```python
from build123d import *

# Parameters (mm, degrees)
SQUARE_FLANGE_SKETCH_70X70_W            = 70
SQUARE_FLANGE_SKETCH_70X70_H            = 70
SQUARE_MOUNTING_FLANGE_DEPTH            = 10
SQUARE_FLANGE_CORNER_FILLETS_R10_R      = 10
SQUARE_FLANGE_HOLES_SKETCH_R            = 5
SQUARE_FLANGE_MOUNTING_HOLES_4X_DEPTH   = 10
ROUND_FLANGE_HOLE_SKETCH_R              = 6
ROUND_FLANGE_BOLT_HOLE_12_DEPTH         = 229.350607619
ROUND_FLANGE_BOLT_HOLE_PATTERN_4X_COUNT = 4


with BuildPart() as part:
    # Housing Profile Sketch → Housing Body Revolve (revolve)
    with BuildSketch(Plane.XY, mode=Mode.PRIVATE) as housing_body_revolve_sk:
        Polygon((0, 15), (43, 15), (43, 30), (202, 30), (202, 60), (222, 60), (222, 24), (49, 24), (49, 9), (0, 9), align=None)
    revolve(housing_body_revolve_sk.sketch.rotate(Axis((0, 0, 0), (1, 0, 0)), 90), axis=Axis((0, 0, 0), (1, 0, 0)))

    # Square Flange Sketch 70x70 → Square Mounting Flange (add)
    with BuildSketch(Plane.ZY):
        Rectangle(SQUARE_FLANGE_SKETCH_70X70_W, SQUARE_FLANGE_SKETCH_70X70_H)
    extrude(amount=SQUARE_MOUNTING_FLANGE_DEPTH)

    # Square Flange Corner Fillets R10
    square_flange_corner_fillets_r10_edges = [part.edges().sort_by_distance(p)[0] for p in [
        (-5, -35, 35),
        (-5, 35, 35),
        (-5, 35, -35),
        (-5, -35, -35),
    ]]
    fillet(square_flange_corner_fillets_r10_edges, radius=SQUARE_FLANGE_CORNER_FILLETS_R10_R)

    # Square Flange Holes Sketch → Square Flange Mounting Holes 4x (cut)
    with BuildSketch(Plane.ZY.offset(10)):
        with Locations((25, 25)):
            Circle(SQUARE_FLANGE_HOLES_SKETCH_R)
        with Locations((-25, 25)):
            Circle(SQUARE_FLANGE_HOLES_SKETCH_R)
        with Locations((-25, -25)):
            Circle(SQUARE_FLANGE_HOLES_SKETCH_R)
        with Locations((25, -25)):
            Circle(SQUARE_FLANGE_HOLES_SKETCH_R)
    extrude(amount=-SQUARE_FLANGE_MOUNTING_HOLES_4X_DEPTH, mode=Mode.SUBTRACT)

    # Round Flange Hole Sketch → Round Flange Bolt Hole Ø12 (cut, through all)
    with BuildSketch(Plane.ZY.offset(-202)):
        with Locations((45, 0)):
            Circle(ROUND_FLANGE_HOLE_SKETCH_R)
    round_flange_bolt_hole_12 = extrude(amount=-ROUND_FLANGE_BOLT_HOLE_12_DEPTH, mode=Mode.SUBTRACT)

    # Round Flange Bolt Hole Pattern 4x: Round Flange Bolt Hole Ø12 ×4 about axis
    round_flange_bolt_hole_pattern_4x_axis = Axis((0, 0, 0), (1, 0, 0))
    for i in range(1, ROUND_FLANGE_BOLT_HOLE_PATTERN_4X_COUNT):
        add(round_flange_bolt_hole_12.rotate(round_flange_bolt_hole_pattern_4x_axis, i * 360 / ROUND_FLANGE_BOLT_HOLE_PATTERN_4X_COUNT), mode=Mode.SUBTRACT)


solid = part.part
```
Here's how the part is built. I have some questions about the finished solid (model axes, mm). A direction names the side the tool comes from. Coordinates: 2 decimals unless noted, no trailing zeros. Loops run counter-clockwise (first coordinate to the right, second up) from the corner with the lowest first, then second, coordinate; pieces in that order, holes last. Notation, with made-up numbers: (81, -32) - (116, -32) arc R30 ccw to (116, 3) - close; hole circle Ø9 at (88, 38). An arc over 180 degrees is marked (long way). Answer as CSV lines item,"result".
Q1. If we section it at A-A, the plane y = 0: Give the number of separate pieces and of enclosed holes in the cut face, and give its area (3 significant figures).
Response:
separate pieces,"3"
enclosed holes,"0"
area,"4,260 mm2"
Q2. If we section it at C-C, the plane y = 45: Write out the boundary of the cut face in (x, z), and give its area (3 significant figures).
Response:
outline,"(202, -39.69) - (222, -39.69) - (222, -6) - (202, -6) - close; (202, 6) - (222, 6) - (222, 39.69) - (202, 39.69) - close"
area,"1,350 mm2"
Q3. We'd pull the mould along Y, two halves only. Please class faces 6 (the face through (21.8, -12.65, 8.06)), 7 (the face through (-5.07, 20.12, 23.92)), 8 (the face through (-5, 35, 0)): pulls with the +Y half, pulls with the -Y half, needs draft (parallel to the pull), parting line crosses it, or undercut.
Response:
face 6,"parting line crosses it"
face 7,"undercut"
face 8,"pulls with the +Y half"
Q4. For pin 1 (5 mm diameter, centred on x = -3, y = -6.5, fed in from -Z); pin 2 (10 mm diameter, centred on x = 161.5, z = 11.5, fed in from -Y); pin 3 (3 mm diameter, centred on x = -3.5, y = 6.5, fed in from +Z); pin 4 (11 mm diameter, centred on y = 0, z = 45, fed in from +X), each with a flat end and sliding along its axis, tell me the tip position at first contact or that it passes through.
Response:
pin 1,"z = -35"
pin 2,"y = -29.29"
pin 3,"z = 35"
pin 4,"through"
Q5. If I drill on L1, parallel to Y at x = -2.25, z = -25; L2, parallel to X at y = 24.5, z = -15.5; L3, parallel to X at y = 3, z = -6, over which ranges is the centre line in solid material (lowest first)? Write a range as [from, to].
Response:
L1,"[-35, -30], [-20, 20], [30, 35]"
L2,"[-10, 0], [43, 222]"
L3,"[-10, 0]"
Q6. For faces 1 (the face through (0, 16, 0)), 2 (the face through (24.157, -6.083, -6.633)), 3 (the face through (-5.07, 31.99, -32.15)), 4 (the face through (-5.07, -32.15, 31.99)), 5 (the face through (-5, -35, 0)), which set-ups out of +Z, -Z, +X, -X, +Y, -Y let a thin tool reach every point of the face, with its end or its side?
Response:
face 1,"none"
face 2,"+X"
face 3,"-Z, -X, +Y"
face 4,"+Z, -X, -Y"
face 5,"+Z, -Z, -X, -Y"
